```python
from build123d import *

# Parameters (mm, degrees)
SKETCH_2_R      = 7
EXTRUDE_1_DEPTH = 10
EXTRUDE_2_DEPTH = 8
SKETCH_4_R      = 8
EXTRUDE_3_DEPTH = 120


with BuildPart() as part:
    # 草图1 → 旋转1 (revolve)
    with BuildSketch(Plane.XY, mode=Mode.PRIVATE) as revolve_1_sk:
        Polygon((0, 30), (0, 0), (50, 0), (50, 10), (15, 30), align=None)
    revolve(revolve_1_sk.sketch.rotate(Axis((0, 30, 0), (0, -1, 0)), 180), axis=Axis((0, 30, 0), (0, -1, 0)))

    # 草图2 → 凸台-拉伸1 (add)
    with BuildSketch(Plane(origin=(0, 30, 0), x_dir=(1, 0, 0), z_dir=(0, 1, 0))):
        Circle(SKETCH_2_R)
    extrude(amount=EXTRUDE_1_DEPTH)

    # 草图3 → 凸台-拉伸2 (add)
    with BuildSketch(Plane(origin=(0, 40, 0), x_dir=(1, 0, 0), z_dir=(0, 1, 0))):
        Polygon((0, 12.124355653), (-10.5, 6.062177826), (-10.5, -6.062177826), (0, -12.124355653), (10.5, -6.062177826), (10.5, 6.062177826), align=None)
    extrude(amount=EXTRUDE_2_DEPTH)

    # 草图4 → 凸台-拉伸3 (add)
    with BuildSketch(Plane(origin=(0, 48, 0), x_dir=(1, 0, 0), z_dir=(0, 1, 0))):
        with Locations(Location((0, 0, 0), (0, 0, 270))):
            Circle(SKETCH_4_R)
    extrude(amount=EXTRUDE_3_DEPTH)


solid = part.part
```
Can you work these out from the model? Positions are in its coordinate system, mm. A direction names the side the tool comes from. Coordinates: 2 decimals unless noted, no trailing zeros. Write each loop counter-clockwise with the first axis right and the second up, starting at its lowest first coordinate (ties: lowest second). Pieces come first, ordered by that corner, then holes. Notation, with made-up numbers: (-13, 86.5) - (-3, 86.5) arc R22 ccw to (-3, 111.5) - close; hole circle Ø7 at (48, 74.5). An arc over 180 degrees is marked (long way). Return JSON: item names as keys, results as strings.
Q1. Thinking about a two-plate mould opening in Y: for faces 1 (the flat face through (-5.324, 43.944, 9.051)), 2 (the flat face through (-3.1, 30, 6.5)), 3 (the conical face through (-15.928, 29.029, -5.016)), which applies, +Y half, -Y half, draft (parallel to the pull), parting line (faces both ways), or undercut?
Computed values:
{"face 1": "draft", "face 2": "undercut", "face 3": "+Y half"}
Q2. If we section it at B-B (y = 36): Please give me the cut outline in (x, z), then the cut area to 3 significant figures.
Computed values:
{"outline": "circle Ø14 at (0, 0)", "area": "154 mm2"}
Q3. On a 3-axis mill with a long thin cutter (end or side, diameter ignored), from which of +Z, -Z, +X, -X, +Y, -Y can I reach the whole of each face in a straight line? I mean faces 4 (the flat face through (-7.15, 40, -0.17)), 5 (the cylindrical face through (-7.81, 107.16, -1.73)), 6 (the flat face through (5.176, 43.944, 9.136)). Say none if no direction works.
Computed values:
{"face 4": "none", "face 5": "+Y", "face 6": "+Z, +X, +Y"}
Q4. I'm going to push flat-ended pins straight in: pin 1 Ø5 at (y, z) = (25.5, 5) entering from -X; pin 2 Ø8 at (x, z) = (-11.5, -8) entering from +Y; pin 3 Ø9 at (y, z) = (43, 0.5) entering from +X. Where does each tip first touch, or does it pass through?
Computed values:
{"pin 1": "stops at x = -26.81", "pin 2": "stops at y = 48", "pin 3": "stops at x = 10.5"}
Q5. If we section it at A-A (z = 0): Please give me the cut outline in (x, y).
Computed values:
{"outline": "(-50, 0) - (50, 0) - (50, 10) - (15, 30) - (7, 30) - (7, 40) - (10.5, 40) - (10.5, 48) - (8, 48) - (8, 168) - (-8, 168) - (-8, 48) - (-10.5, 48) - (-10.5, 40) - (-7, 40) - (-7, 30) - (-15, 30) - (-50, 10) - close"}
Q6. Please list where these lines run through material, in increasing order: L1, parallel to Y at x = -42.5, z = 18.5; L2, parallel to Y at x = 34.5, z = -2.5; L3, parallel to X at y = 44, z = 11.5. Write a range as from..to.
Computed values:
{"L1": "y = 0..12.08", "L2": "y = 0..18.81", "L3": "x = -1.08..1.08"}
Q7. If we section it at C-C (y = 79): Please give me the cut outline in (x, z).
Computed values:
{"outline": "circle Ø16 at (0, 0)"}
